Could you check a few things on this drawing? It's one solid part, dimensions in mm from its lowest x, y, z. Round coordinates to 2 decimals unless told otherwise and drop trailing zeros. Order: outer loops, then holes, each group sorted by start corner. A loop starts at its lowest first (then second) coordinate and runs counter-clockwise, first axis right, second up. Notation, with made-up numbers: (77, 43.5) -> (90, 43.5) arc R33 ccw to (90, 82.5) -> close; hole circle Ø10 at (12, 53.5). An arc over 180 degrees is marked (long way). Use a Markdown table: item, result. Add a question column.
(1) If I drill on probe 1 along Z at (x, y) = (352, 26.5); probe 2 along Z at (x, y) = (155.5, 14.5); probe 3 along X at (y, z) = (17.5, 50.5), over which ranges is the centre line in solid material (lowest first)?
(2) I want a section at B-B, the plane x = 76. Please give me the cut outline in (y, z).
(3) I'm going to push flat-ended pins straight in: P1, Ø10, axis at y = 25, z = 52.5, coming from the +X side; P2, Ø1, axis at x = 255.5, y = 12.5, coming from the -Z side; P3, Ø5, axis at y = 10, z = 53.5, coming from the +X side. Where does each tip first touch, or does it pass through?
(4) I want a section at C-C, the plane z = 16.5. Please give me the cut outline in (x, y).
(5) I want a section at A-A, the plane y = 7.5. Please give me the cut outline in (x, z), then the cut area to 3 significant figures.
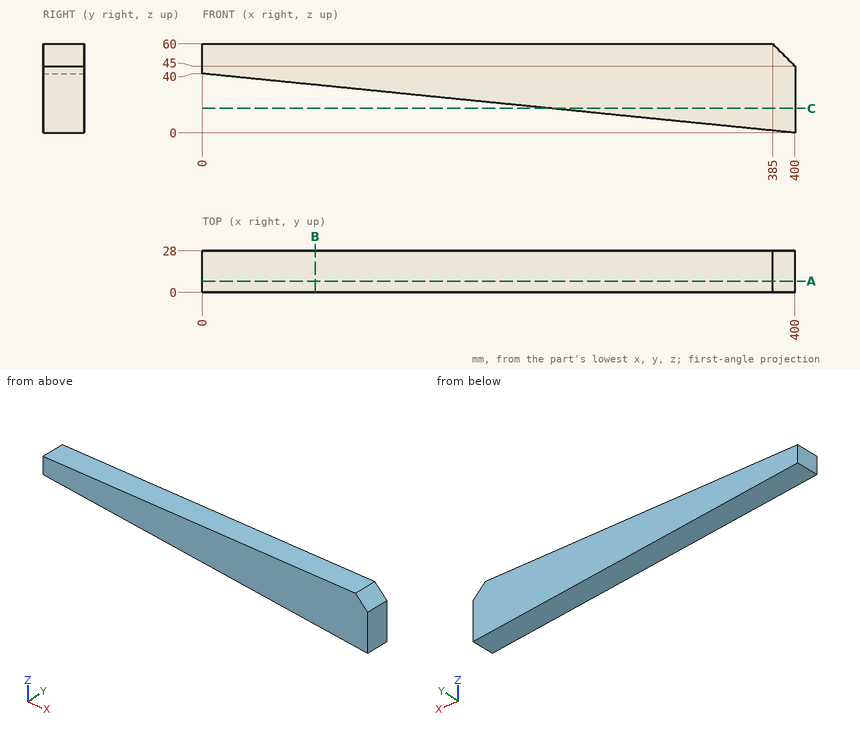
Taken from the geometry:
| question | item | result |
|---|---|---|
| 1 | probe 1 | z = 4.8 to 60 |
| 1 | probe 2 | z = 24.45 to 60 |
| 1 | probe 3 | x = 0 to 394.5 |
| 2 | outline | (0, 32.4) -> (28, 32.4) -> (28, 60) -> (0, 60) -> close |
| 3 | P1 | stops at x = 397.5 |
| 3 | P2 | stops at z = 14.4 |
| 3 | P3 | stops at x = 394 |
| 4 | outline | (235, 0) -> (400, 0) -> (400, 28) -> (235, 28) -> close |
| 5 | outline | (0, 40) -> (400, 0) -> (400, 45) -> (385, 60) -> (0, 60) -> close |
| 5 | area | 15,900 mm2 |
